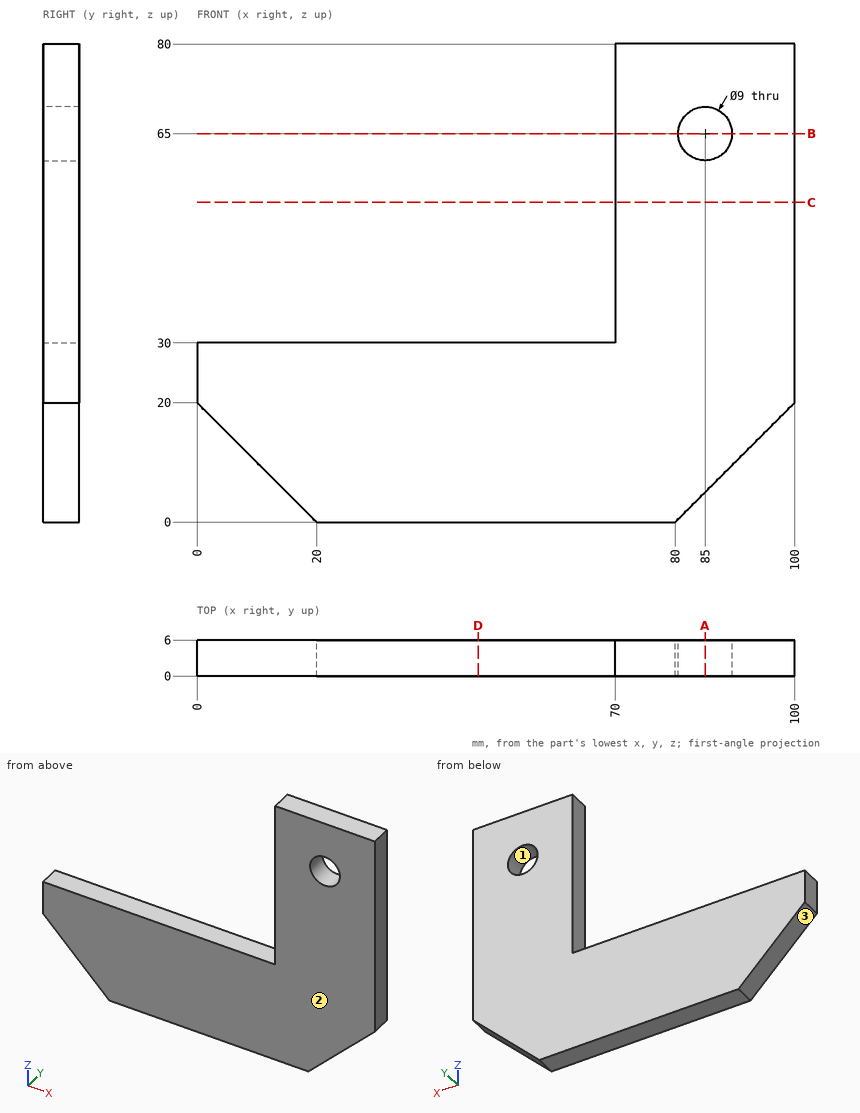
Source: three-view drawing plus pictorial views. Frame: mm from the lowest corner of the part. Coordinates: 2 decimals unless noted, no trailing zeros. Write each loop counter-clockwise with the first axis right and the second up, starting at its lowest first coordinate (ties: lowest second). Pieces come first, ordered by that corner, then holes. Notation, with made-up numbers: (23.5, -13) -> (29.5, -13) arc R13 cw to (29.5, -8) -> close; hole circle Ø10 at (-19.75, 38). An arc over 180 degrees is marked (long way). Answer as a JSON object with one key per item and string values.
1. Section D-D on x = 47. Return the cut outline in (y, z), then the cut area to 3 significant figures.
Result set:
{"outline": "(0, 0) -> (6, 0) -> (6, 30) -> (0, 30) -> close", "area": "180 mm2"}
2. Section B-B on z = 65. Return the cut outline in (x, y), then the cut area to 3 significant figures.
Result set:
{"outline": "(70, 0) -> (80.5, 0) -> (80.5, 6) -> (70, 6) -> close; (89.5, 0) -> (100, 0) -> (100, 6) -> (89.5, 6) -> close", "area": "126 mm2"}
3. Material intervals for line 1 (X direction, y = 1.9, z = 65); line 2 (Z direction, x = 64, y = 5.25); line 3 (X direction, y = 1.5, z = 39.5), sorted ascending. Write a range as from..to.
Result set:
{"line 1": "x = 70..80.5, 89.5..100", "line 2": "z = 0..30", "line 3": "x = 70..100"}
4. Section A-A on x = 85. Return the cut outline in (y, z).
Result set:
{"outline": "(0, 5) -> (6, 5) -> (6, 60.5) -> (0, 60.5) -> close; (0, 69.5) -> (6, 69.5) -> (6, 80) -> (0, 80) -> close"}
5. First-contact query: P1, Ø1.5, axis at y = 5, z = 18.5, coming from the -X side; P2, Ø2, axis at y = 4, z = 71.5, coming from the -X side. Flat tips, straight axial feed; report the tip coordinate or a pass-through.
Result set:
{"P1": "stops at x = 0.75", "P2": "stops at x = 70"}
6. Section C-C on z = 53.5. Return the cut outline in (x, y).
Result set:
{"outline": "(70, 0) -> (100, 0) -> (100, 6) -> (70, 6) -> close"}
7. Mould query, pull axis Z, two halves, no side actions, for the marked faces 1, 2 and 3. Classes: released by +Z, released by -Z, zero draft, split by the parting line, or undercut.
Result set:
{"face 1": "undercut", "face 2": "zero draft", "face 3": "released by -Z"}
